Could you check a few things on this model? Use its own coordinates, in mm. Face numbers are marked on the shaded views. A direction names the side the tool comes from. Round coordinates to 2 decimals unless told otherwise and drop trailing zeros. Loops run counter-clockwise (first coordinate to the right, second up) from the corner with the lowest first, then second, coordinate; pieces in that order, holes last. Notation, with made-up numbers: M 87.25,37 L 136.25,37 A25 ccw 136.25,69 Z; hole C 57.25,43 d5. An arc over 180 degrees is marked long. Answer in a Markdown table with one row per item.
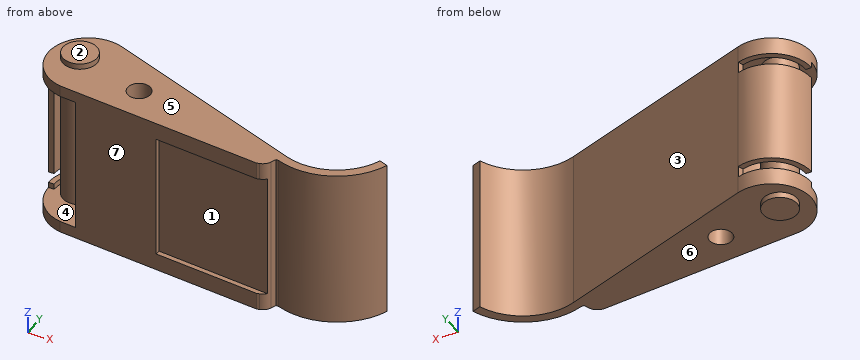
```python
from build123d import *

# Parameters (mm, degrees)
EXTRUDE_1_DEPTH          = 7
EXTRUDE_1_DEPTH_BACK     = 7
SKETCH_1_R               = 1
CUT_EXTRUDE_1_DEPTH      = 6
CUT_EXTRUDE_1_DEPTH_BACK = 6
CUT_EXTRUDE_2_DEPTH      = 6
CUT_EXTRUDE_2_DEPTH_BACK = 6
SKETCH_3_R               = 3
CUT_EXTRUDE_START        = -1
CUT_EXTRUDE_3_DEPTH      = 1
CUT_EXTRUDE_4_DEPTH      = 1
EXTRUDE_2_DEPTH          = 7.5
EXTRUDE_2_DEPTH_BACK     = 7.5
SKETCH_6_R               = 1.5
CUT_EXTRUDE_5_DEPTH      = 5.5
CUT_EXTRUDE_5_DEPTH_BACK = 5.5


with BuildPart() as part:
    # 草图1 → 凸台-拉伸1 (new, two sides: drawn at the far end of the back side and taken through both)
    with BuildSketch(Plane.XY.offset(-EXTRUDE_1_DEPTH_BACK)):
        with BuildLine():
            Line((2.892231378, 2.053172864), (21, 0.468948388))
            Line((21, 0.468948388), (21.243569075, 0.530116447))
            ThreePointArc((21.243569075, 0.530116447), (21.657311704, 0.746381181), (21.927791013, 1.126899697))
            Line((21.927791013, 1.126899697), (22.11, 1.58))
            Line((22.11, 1.58), (22.31866709, 1.58))
            ThreePointArc((22.31866709, 1.58), (26.857258232, 1.7173207), (30, 4.994642886))
            Line((30, 4.994642886), (29.24792212, 5.268376848))
            ThreePointArc((29.24792212, 5.268376848), (26.549597889, 2.45607622), (22.654950899, 2.308721878))
            Line((22.654950899, 2.308721878), (4.688013818, 8.792206429))
            ThreePointArc((4.688013818, 8.792206429), (0.118016194, 6.401213367), (2.892231378, 2.053172864))
        make_face()
        with Locations((8.57, 4.38)):
            Circle(SKETCH_1_R, mode=Mode.SUBTRACT)
    extrude(amount=EXTRUDE_1_DEPTH + EXTRUDE_1_DEPTH_BACK)

    # 草图2 → 切除-拉伸1 (cut, two sides: drawn at the far end of the back side and taken through both)
    with BuildSketch(Plane.XY.offset(-CUT_EXTRUDE_1_DEPTH_BACK)):
        with BuildLine():
            Line((4.63, 0.629363491), (3.5, 5.5))
            Line((3.5, 5.5), (-1.5, 5.5))
            ThreePointArc((-1.5, 5.5), (0.389533797, 1.585284174), (4.63, 0.629363491))
        make_face()
    extrude(amount=CUT_EXTRUDE_1_DEPTH + CUT_EXTRUDE_1_DEPTH_BACK, mode=Mode.SUBTRACT)

    # 草图3 → 切除-拉伸2 (cut, two sides: drawn at the far end of the back side and taken through both)
    with BuildSketch(Plane.XY.offset(-CUT_EXTRUDE_2_DEPTH_BACK)):
        with Locations((3.5, 5.5)):
            Circle(SKETCH_3_R)
    extrude(amount=CUT_EXTRUDE_2_DEPTH + CUT_EXTRUDE_2_DEPTH_BACK, mode=Mode.SUBTRACT)

    # 草图4 → 切除-拉伸3 (cut)
    with BuildSketch(Plane.XY.offset(5.5).offset(CUT_EXTRUDE_START)):
        with BuildLine():
            Line((2.360511459, 2.190684985), (4.639488541, 8.809315015))
            ThreePointArc((4.639488541, 8.809315015), (0.190684985, 6.639488541), (2.360511459, 2.190684985))
        make_face()
    extrude(amount=CUT_EXTRUDE_3_DEPTH, mode=Mode.SUBTRACT)

    # 草图5 → 切除-拉伸4 (cut)
    with BuildSketch(Plane.XY.offset(-5.5)):
        with BuildLine():
            Line((2.360511459, 2.190684985), (4.639488541, 8.809315015))
            ThreePointArc((4.639488541, 8.809315015), (0.190684985, 6.639488541), (2.360511459, 2.190684985))
        make_face()
    extrude(amount=CUT_EXTRUDE_4_DEPTH, mode=Mode.SUBTRACT)

    # 草图6 → 凸台-拉伸2 (add, two sides: drawn at the far end of the back side and taken through both)
    with BuildSketch(Plane.XY.offset(-EXTRUDE_2_DEPTH_BACK)):
        with Locations((2.5, 6)):
            Circle(SKETCH_6_R)
    extrude(amount=EXTRUDE_2_DEPTH + EXTRUDE_2_DEPTH_BACK)

    # 草图7 → 切除-拉伸5 (cut, two sides: drawn at the far end of the back side and taken through both)
    with BuildSketch(Plane.XY.offset(-CUT_EXTRUDE_5_DEPTH_BACK)):
        Polygon((11.724964743, 1.0104331), (21.686911724, 0.138875672), (21.747920744, 0.836211961), (11.785973763, 1.707769388), align=None)
    extrude(amount=CUT_EXTRUDE_5_DEPTH + CUT_EXTRUDE_5_DEPTH_BACK, mode=Mode.SUBTRACT)


solid = part.part
```
1) If we mould it in two halves opening along Z, with no side actions, what happens to the marked faces 4, 5, 6 and 7? For each: released by +Z, released by -Z, zero draft, split by the parting line, or undercut.
Computed:
| item | result |
|---|---|
| face 4 | undercut |
| face 5 | released by +Z |
| face 6 | released by -Z |
| face 7 | zero draft |
2) I want a section at A-A, the plane x = 8.57. Please give me the cut outline in (y, z), plus the area to 3 significant figures.
Computed:
| item | result |
|---|---|
| outline | M 1.56,-7 L 3.38,-7 L 3.38,7 L 1.56,7 Z; M 5.38,-7 L 7.39,-7 L 7.39,7 L 5.38,7 Z |
| area | 53.7 mm² |
3) I want a section at B-B, the plane x = 2.5. Please give me the cut outline in (y, z), plus the area to 3 significant figures.
Computed:
| item | result |
|---|---|
| outline | M 2.15,-7 L 4.5,-7 L 4.5,-7.5 L 7.5,-7.5 L 7.5,-7 L 8.85,-7 L 8.85,-5.5 L 8.33,-5.5 L 8.33,-6 L 7.5,-6 L 7.5,6 L 8.33,6 L 8.33,5.5 L 8.85,5.5 L 8.85,7 L 7.5,7 L 7.5,7.5 L 4.5,7.5 L 4.5,7 L 2.15,7 L 2.15,6 L 4.5,6 L 4.5,-6 L 2.15,-6 Z; M 8.33,-4.5 L 8.85,-4.5 L 8.85,4.5 L 8.33,4.5 Z |
| area | 57.7 mm² |
4) I need wall thicknesses on line 1 (Z direction, x = 6, y = 4.5); line 2 (Z direction, x = 7.5, y = 3.75); line 3 (Y direction, x = 5, z = 0.25). Which ranges of each line are inside material? Lowest first, please.
Computed:
| item | result |
|---|---|
| line 1 | z = -7 to -6, 6 to 7 |
| line 2 | z = -7 to 7 |
| line 3 | y = 1.87 to 2.9, 8.1 to 8.68 |
5) Will these pins go through, and if not, where does the flat tip stop? P1, Ø1, axis at x = 17.5, y = 1, coming from the -Z side; P2, Ø4, axis at y = 8, z = 4.5, coming from the -X side; P3, Ø4.5, axis at x = 15.5, y = 4.5, coming from the +Z side; P4, Ø8, axis at x = 22.5, z = 2, coming from the -Y side.
Computed:
| item | result |
|---|---|
| P1 | stops at z = -7 |
| P2 | stops at x = 0.04 |
| P3 | stops at z = 7 |
| P4 | stops at y = 0.47 |
6) I want a section at C-C, the plane x = 20.5. Please give me the cut outline in (y, z), plus the area to 3 significant figures.
Computed:
| item | result |
|---|---|
| outline | M 0.51,-7 L 3.09,-7 L 3.09,7 L 0.51,7 L 0.51,5.5 L 0.95,5.5 L 0.95,-5.5 L 0.51,-5.5 Z |
| area | 31.3 mm² |
7) Which directions (+Z, -Z, +X, -X, +Y, -Y) give clear straight access to the entire face, cutting with the end or side of a thin tool? Please do the marked faces 1, 2 and 3.
Computed:
| item | result |
|---|---|
| face 1 | -Y |
| face 2 | +Z, +X, -X, +Y, -Y |
| face 3 | +Z, -Z, +Y |
